```python
from build123d import *

# Parameters (mm, degrees)
SKETCH1_R           = 1.25
BOSS_EXTRUDE1_DEPTH = 5.5
SKETCH2_R           = 1.75
BOSS_EXTRUDE2_DEPTH = 1.5
CUT_EXTRUDE1_DEPTH  = 0.3


with BuildPart() as part:
    # Sketch1 → Boss-Extrude1 (new body)
    with BuildSketch(Plane(origin=(0, 0, 0), x_dir=(1, 0, 0), z_dir=(0, 1, 0))):
        with Locations(Location((0, 0, 0), (0, 0, 270))):
            Circle(SKETCH1_R)
    extrude(amount=BOSS_EXTRUDE1_DEPTH)

    # Sketch2 → Boss-Extrude2 (add)
    with BuildSketch(Plane(origin=(0, 5.5, 0), x_dir=(1, 0, 0), z_dir=(0, 1, 0))):
        with Locations(Location((0, 0, 0), (0, 0, 270))):
            Circle(SKETCH2_R)
    extrude(amount=BOSS_EXTRUDE2_DEPTH)

    # Sketch3 → Cut-Extrude1 (cut)
    with BuildSketch(Plane(origin=(0, 7, 0), x_dir=(1, 0, 0), z_dir=(0, 1, 0))):
        Polygon((-1.611781927, -1.775402925), (1.143517474, 2.10766798), (1.611781927, 1.775402925), (-1.143517474, -2.10766798), align=None)
    extrude(amount=-CUT_EXTRUDE1_DEPTH, mode=Mode.SUBTRACT)


solid = part.part
```
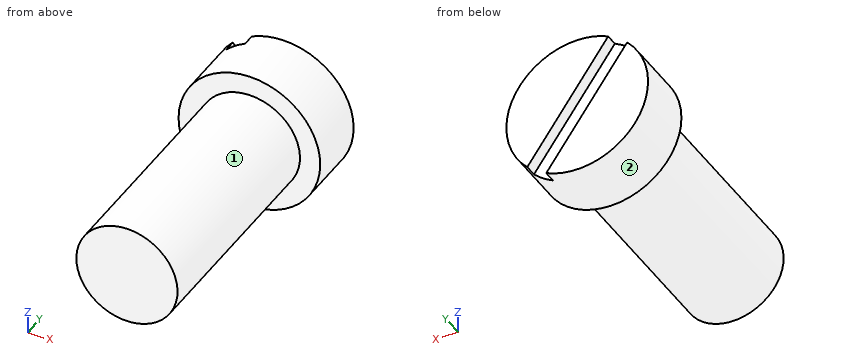
Geometry check sheet. Reference: the model listing, model coordinates, mm. Face numbers are marked on the shaded views. A direction names the side the tool comes from. Coordinates: 2 decimals unless noted, no trailing zeros. Loops run counter-clockwise (first coordinate to the right, second up) from the corner with the lowest first, then second, coordinate; pieces in that order, holes last.
Item 1: Sectioned sample at B-B, the plane z = 0. Record the boundary of the cut face in (x, y), then the cut area to 3 significant figures.
Item 2: Thickness scan on line 1 (Y direction, x = 0.55, z = -0.85); line 2 (Z direction, x = -0.2, y = 5); line 3 (Y direction, x = -1.55, z = 0.55). Record the ranges inside material, lowest first.
Item 3: Access from +Z, -Z, +X, -X, +Y, -Y to the whole of each face (thin tool, end or side, straight path). Record for the marked faces 1 and 2.
Item 4: Sectioned sample at A-A, the plane x = 0.2. Record the boundary of the cut face in (y, z).
Item 5: Go/stop test with a flat-tipped pin: pin 1 Ø1 at (y, z) = (4.5, 0.5) entering from +X. Record where the tip stops, or that it passes through.
Item 6: Sectioned sample at C-C, the plane y = 4.75. Record the boundary of the cut face in (x, z).
Item 7: Sectioned sample at D-D, the plane x = 1. Record the boundary of the cut face in (y, z), then the cut area to 3 significant figures.
Check result:
1. outline: (-1.75, 5.5) - (-1.25, 5.5) - (-1.25, 0) - (1.25, 0) - (1.25, 5.5) - (1.75, 5.5) - (1.75, 7) - (0.35, 7) - (0.35, 6.7) - (-0.35, 6.7) - (-0.35, 7) - (-1.75, 7) - close
1. area: 18.8 mm2
2. line 1: y = 0 to 6.7
2. line 2: z = -1.23 to 1.23
2. line 3: y = 5.5 to 7
3. face 1: -Y
3. face 2: +Y, -Y
4. outline: (0, -1.23) - (5.5, -1.23) - (5.5, -1.74) - (7, -1.74) - (7, -0.78) - (6.7, -0.78) - (6.7, 0.21) - (7, 0.21) - (7, 1.74) - (5.5, 1.74) - (5.5, 1.23) - (0, 1.23) - close
5. pin 1: stops at x = 1.25
6. outline: circle Ø2.5 at (0, 0)
7. outline: (0, -0.75) - (5.5, -0.75) - (5.5, -1.44) - (6.7, -1.44) - (6.7, -0.91) - (7, -0.91) - (7, 1.44) - (5.5, 1.44) - (5.5, 0.75) - (0, 0.75) - close
7. area: 12.4 mm2
